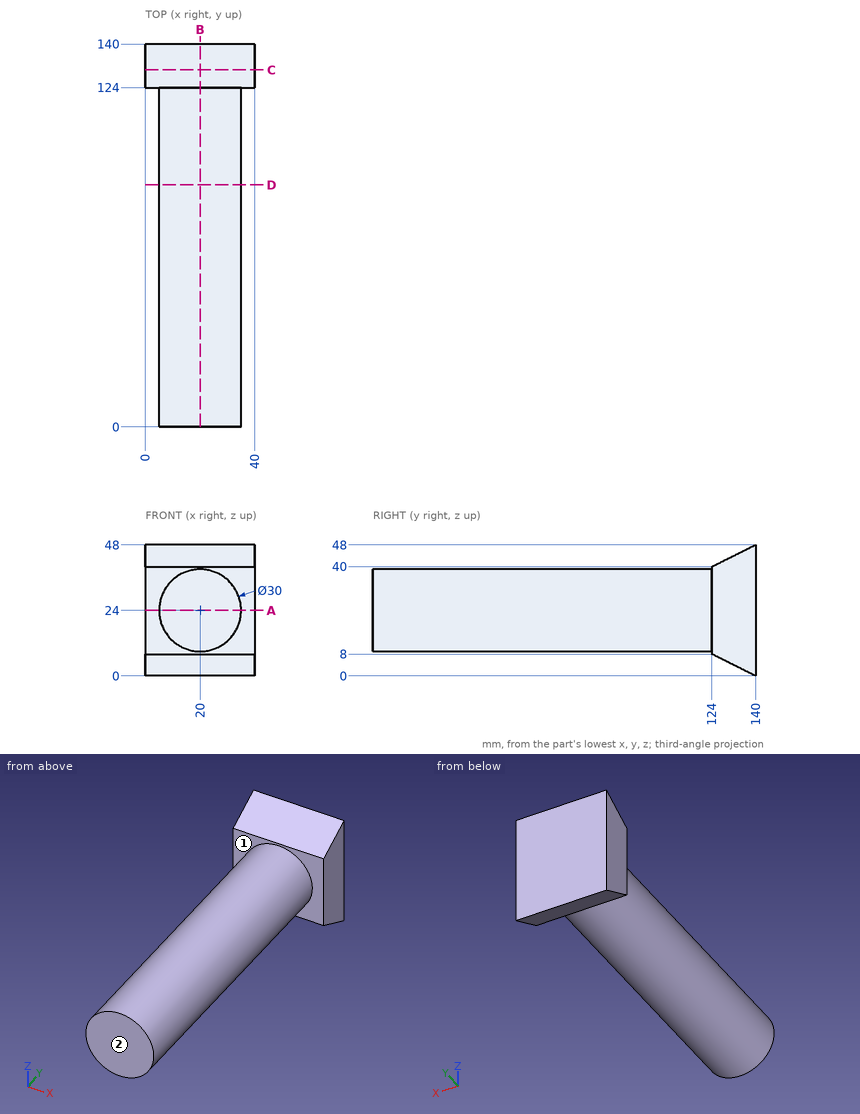
The drawing under review shows one solid part. Ordinate dimensions are in mm from its lowest x, y, z. A direction names the side the tool comes from. Coordinates: 2 decimals unless noted, no trailing zeros. Write each loop counter-clockwise with the first axis right and the second up, starting at its lowest first coordinate (ties: lowest second). Pieces come first, ordered by that corner, then holes. Notation, with made-up numbers: (62, 30.25) - (69, 30.25) arc R17 cw to (69, 42.25) - close; hole circle Ø4 at (-5.75, -27.5). An arc over 180 degrees is marked (long way). Put each result on its own line as item: value.
1. Add section D-D, the plane y = 88.5. Give the boundary of the cut face in (x, z), then the cut area to 3 significant figures.
Values found:
outline: circle Ø30 at (20, 24)
area: 707 mm²
2. Machinability: for the marked faces 1 and 2, which of the approach directions +Z, -Z, +X, -X, +Y, -Y give a long, thin tool a straight path to every point of the face, cutting with its end or side? Answer none if there is none.
Values found:
face 1: -Y
face 2: +Z, -Z, +X, -X, -Y
3. Add section C-C, the plane y = 130.5. Give the boundary of the cut face in (x, z), then the cut area to 3 significant figures.
Values found:
outline: (0, 4.75) - (40, 4.75) - (40, 43.25) - (0, 43.25) - close
area: 1,540 mm²
4. For pin 1 (8 mm diameter, centred on x = 21, y = 100.5, fed in from -Z); pin 2 (12 mm diameter, centred on x = 33, y = 68, fed in from -Z); pin 3 (1 mm diameter, centred on x = 18.5, z = 40, fed in from -Y), all flat-tipped, find the tip position at first contact; note any pin that passes through.
Values found:
pin 1: z = 9
pin 2: z = 10.73
pin 3: y = 124
5. Add section B-B, the plane x = 20. Give the boundary of the cut face in (y, z).
Values found:
outline: (0, 9) - (124, 9) - (124, 8) - (140, 0) - (140, 48) - (124, 40) - (124, 39) - (0, 39) - close
6. Add section A-A, the plane z = 24. Give the boundary of the cut face in (x, y), then the cut area to 3 significant figures.
Values found:
outline: (0, 124) - (5, 124) - (5, 0) - (35, 0) - (35, 124) - (40, 124) - (40, 140) - (0, 140) - close
area: 4,360 mm²
7. Wall thickness on probe 1 along Y at (x, z) = (5, 32); probe 2 along X at (y, z) = (112.5, 22); probe 3 along Z at (x, y) = (9.5, 38): over which ranges is each line inside the solid? List them lowest first.
Values found:
probe 1: 124 to 140
probe 2: 5.13 to 34.87
probe 3: 13.29 to 34.71
